from build123d import *

# Parameters (mm, degrees)
BOSS_EXTRUDE1_DEPTH     = 20
M10X1_25_TAPPED_HOLE1_D = 8.8
HOLE1_D                 = 6.6
HOLE1_CBORE_D           = 11
HOLE1_CBORE_DEPTH       = 10
CHAMFER1_SIZE           = 1


with BuildPart() as part:
    # Sketch1 → Boss-Extrude1 (new body)
    with BuildSketch(Plane.XY):
        Polygon((6.43607117, 42.87394958), (6.43607117, -5.12605042), (-33.56392883, -5.12605042), (-33.56392883, -25.12605042), (26.43607117, -25.12605042), (26.43607117, 42.87394958), align=None)
    extrude(amount=BOSS_EXTRUDE1_DEPTH)

    # M10x1.25 Tapped Hole1 (through all)
    with Locations(Plane.ZY.offset(-6.43607117)):
        with Locations((10, 17.87394958)):
            Hole(M10X1_25_TAPPED_HOLE1_D / 2)

    # Hole1 (through all)
    with Locations(Plane(origin=(0, -5.12605042, 0), x_dir=(1, 0, 0), z_dir=(0, 1, 0))):
        with Locations((-3.56392883, -10), (-23.56392883, -10)):
            CounterBoreHole(HOLE1_D / 2, HOLE1_CBORE_D / 2, HOLE1_CBORE_DEPTH)

    # Chamfer1
    chamfer1_edges = [part.edges().sort_by_distance(p)[0] for p in [
        (26.43607117, 42.87394958, 10),
        (26.43607117, -25.12605042, 10),
        (-33.56392883, -25.12605042, 10),
        (-33.56392883, -5.12605042, 10),
        (6.43607117, 42.87394958, 10),
    ]]
    chamfer(chamfer1_edges, length=CHAMFER1_SIZE)


solid = part.part
Work out the finished part from the listing and answer in its coordinate system (mm). A direction names the side the tool comes from. Round coordinates to 2 decimals unless told otherwise and drop trailing zeros. Order: outer loops, then holes, each group sorted by start corner. A loop starts at its lowest first (then second) coordinate and runs counter-clockwise, first axis right, second up. Notation, with made-up numbers: M 70.5,23 L 118.5,23 A12 cw 118.5,45 Z; hole C 59.5,-23 d11. An arc over 180 degrees is marked long. Put each result on its own line as item: value. Start each with the question number.
Q1. Section B-B, the plane y = 19.5 is taken. Write down the section's boundary in (x, z), and give its area (3 significant figures).
Q2. Section C-C, the plane y = -13 is taken. Write down the section's boundary in (x, z), and give its area (3 significant figures).
Q3. Flat-ended cylindrical pins translate along their axes: pin 1 (11.5 mm diameter, centred on y = 17.87, z = 10, fed in from -X); pin 2 (5.5 mm diameter, centred on x = -3.56, z = 10, fed in from +Y); pin 3 (10 mm diameter, centred on x = -3.5, z = 17.5, fed in from +Y); pin 4 (9 mm diameter, centred on x = -3.56, z = 10, fed in from +Y). Find the tip coordinate at first contact, or state that the pin passes through.
Q4. Straight lines are drawn through the part: L1, parallel to X at y = -21.75, z = 10; L2, parallel to X at y = -18, z = 12.75; L3, parallel to Y at x = 5, z = 5.5. For each, find the intervals that lie inside material, in ascending order. Write a range as [from, to].
Q5. Section D-D, the plane x = 12 is taken. Write down the section's boundary in (y, z).
Q6. A tool of negligible diameter and unlimited length cuts with its end or side. For faces 5 (the cylindrical face through (-4.76, -10.06, 15.37)), 6 (the flat face through (-13, -5.126, 10)), 7 (the flat face through (-4, -25.126, 5)), from which of +Z, -Z, +X, -X, +Y, -Y can it reach the whole face along a straight path? Write none if from no direction.
Q7. For a pull along X with two mould halves and no side action, classify faces 1 (the cylindrical face through (-27.929, -10.056, 13.347)), 2 (the flat face through (-33.564, -15, 10)), 3 (the flat face through (-24, -15.126, 14)), 4 (the flat face through (26.436, 8, 10)) as pulls with the +X half, pulls with the -X half, needs draft (parallel to the pull), parting line crosses it, or undercut.
Q8. Section A-A, the plane z = 10 is taken. Give the number of separate pieces and of enclosed holes in the cut face, and give its area (3 significant figures).
Findings below:
1. outline: M 6.44,0 L 26.44,0 L 26.44,5.91 L 6.44,5.91 Z; M 6.44,14.09 L 26.44,14.09 L 26.44,20 L 6.44,20 Z
1. area: 236 mm^2
2. outline: M -33.56,0 L 26.44,0 L 26.44,20 L -33.56,20 Z; hole C -23.56,10 d11; hole C -3.56,10 d11
2. area: 1,010 mm^2
3. pin 1: stops at x = 6.44
3. pin 2: passes through
3. pin 3: stops at y = -5.13
3. pin 4: stops at y = -15.13
4. L1: x = [-33.56, -26.86], [-20.26, -6.86], [-0.26, 26.44]
4. L2: x = [-33.56, -25.39], [-21.74, -5.39], [-1.74, 26.44]
4. L3: y = [-25.13, -5.13]
5. outline: M -25.13,0 L 42.87,0 L 42.87,20 L -25.13,20 Z; hole C 17.87,10 d8.8
6. face 5: +Y
6. face 6: +Z, -Z, -X, +Y
6. face 7: +Z, -Z, +X, -X, -Y
7. face 1: undercut
7. face 2: pulls with the -X half
7. face 3: undercut
7. face 4: pulls with the +X half
8. separate pieces: 4
8. enclosed holes: 0
8. area: 1,630 mm^2
